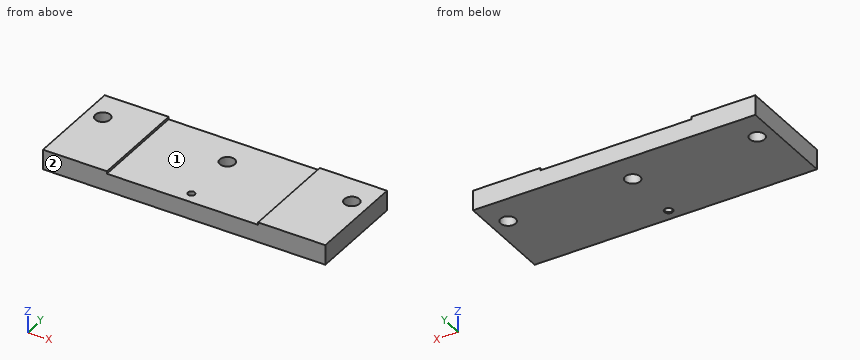
from build123d import *

# Parameters (mm, degrees)
SKETCH_1_W                   = 170
SKETCH_1_H                   = 60
SKETCH_1_R                   = 4.5
EXTRUDE_1_DEPTH              = 6
SKETCH_2_W                   = 91
SKETCH_2_H                   = 60
CUT_EXTRUDE_1_DEPTH          = 1.5
HOLE_WIZARD_M5_1_D           = 4.2
HOLE_WIZARD_M5_1_CSINK_D     = 5.05
HOLE_WIZARD_M5_1_CSINK_ANGLE = 90


with BuildPart() as part:
    # 草图1 → 凸台-拉伸1 (new, symmetric)
    with BuildSketch(Plane.XY):
        Rectangle(SKETCH_1_W, SKETCH_1_H)
        with Locations((-75, 12)):
            Circle(SKETCH_1_R, mode=Mode.SUBTRACT)
        with Locations((75, 12)):
            Circle(SKETCH_1_R, mode=Mode.SUBTRACT)
        with Locations((0, 12)):
            Circle(SKETCH_1_R, mode=Mode.SUBTRACT)
    extrude(amount=EXTRUDE_1_DEPTH, both=True)

    # 草图2 → 切除-拉伸1 (cut)
    with BuildSketch(Plane.XY.offset(6)):
        with Locations((-1, 0)):
            Rectangle(SKETCH_2_W, SKETCH_2_H)
    extrude(amount=-CUT_EXTRUDE_1_DEPTH, mode=Mode.SUBTRACT)

    # M5 螺纹孔1 (through all)
    with Locations(Plane(origin=(0, -23, -6), x_dir=(-1, 0, 0), z_dir=(0, 0, -1))):
        with Locations((0, 0)):
            CounterSinkHole(HOLE_WIZARD_M5_1_D / 2, HOLE_WIZARD_M5_1_CSINK_D / 2, counter_sink_angle=HOLE_WIZARD_M5_1_CSINK_ANGLE)


solid = part.part
The model under review builds one solid part; all positions refer to its coordinate system, in mm. Face numbers are marked on the shaded views. Round coordinates to 2 decimals unless told otherwise and drop trailing zeros. Loops run counter-clockwise (first coordinate to the right, second up) from the corner with the lowest first, then second, coordinate; pieces in that order, holes last. Notation, with made-up numbers: (-6, 24.25) -> (11, 24.25) arc R36 cw to (11, 62.25) -> close; hole circle Ø4 at (86.25, -1). An arc over 180 degrees is marked (long way). Write item = value, one per line. Start each with the question number.
Item 1: Take a section at B-B on x = 75. Give the boundary of the cut face in (y, z), plus the area to 3 significant figures.
Item 2: Mouldability with a two-part tool opening along X and no side actions: class the marked faces 1 and 2 as released by +X, released by -X, zero draft, split by the parting line, or undercut.
Item 3: To check wall thickness, follow L1, parallel to Y at x = 0, z = 0; L2, parallel to Y at x = -75, z = 1.5; L3, parallel to X at y = -23, z = 1. State the ranges of each line that lie inside material, in increasing order.
Item 4: Insertion check: pin 1 (18 mm diameter, centred on x = 11.5, y = 1, fed in from +Z); pin 2 (5 mm diameter, centred on x = 0, y = -23, fed in from -Z) (3 decimals). Each pin has a flat end and moves straight along its axis. Give the tip position at first contact, or say it passes through.
Item 5: Take a section at A-A on z = -1.25. Give the boundary of the cut face in (x, y), plus the area to 4 significant figures.
Item 6: Take a section at C-C on y = -23. Give the boundary of the cut face in (x, z) (3 decimals), plus the area to 3 significant figures.
Item 7: Take a section at D-D on x = 0. Give the boundary of the cut face in (y, z) (3 decimals), plus the area to 3 significant figures.
Result:
q1.outline = (-30, -6) -> (7.5, -6) -> (7.5, 6) -> (-30, 6) -> close; (16.5, -6) -> (30, -6) -> (30, 6) -> (16.5, 6) -> close
q1.area = 612 mm²
q2.face_1 = undercut
q2.face_2 = zero draft
q3.L1 = -30 to -25.1, -20.9 to 7.5, 16.5 to 30
q3.L2 = -30 to 7.5, 16.5 to 30
q3.L3 = -85 to -2.1, 2.1 to 85
q4.pin_1 = 4.5
q4.pin_2 = -5.975
q5.outline = (-85, -30) -> (85, -30) -> (85, 30) -> (-85, 30) -> close; hole circle Ø9 at (-75, 12); hole circle Ø9 at (0, 12); hole circle Ø4.2 at (0, -23); hole circle Ø9 at (75, 12)
q5.area = 10,000 mm²
q6.outline = (-85, -6) -> (-2.525, -6) -> (-2.1, -5.575) -> (-2.1, 4.5) -> (-46.5, 4.5) -> (-46.5, 6) -> (-85, 6) -> close; (2.1, -5.575) -> (2.525, -6) -> (85, -6) -> (85, 6) -> (44.5, 6) -> (44.5, 4.5) -> (2.1, 4.5) -> close
q6.area = 1,860 mm²
q7.outline = (-30, -6) -> (-25.525, -6) -> (-25.1, -5.575) -> (-25.1, 4.5) -> (-30, 4.5) -> close; (-20.9, -5.575) -> (-20.475, -6) -> (7.5, -6) -> (7.5, 4.5) -> (-20.9, 4.5) -> close; (16.5, -6) -> (30, -6) -> (30, 4.5) -> (16.5, 4.5) -> close
q7.area = 491 mm²
